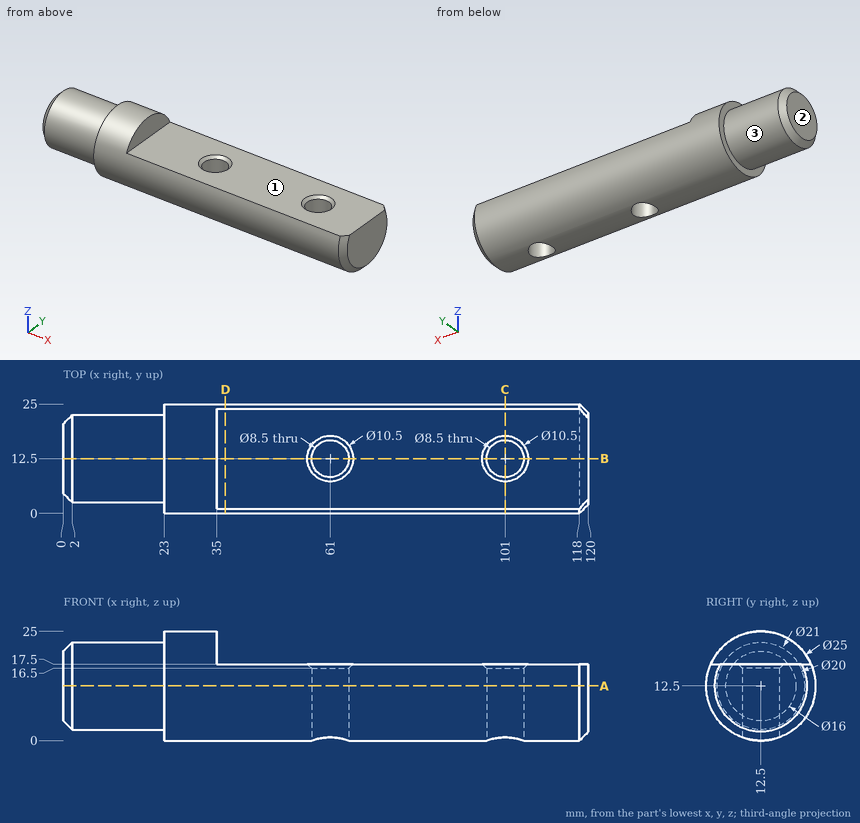
Here's the drawing with two shaded views (mm, measured from the low corner). I have some questions. A direction names the side the tool comes from. Coordinates: 2 decimals unless noted, no trailing zeros. Write each loop counter-clockwise with the first axis right and the second up, starting at its lowest first coordinate (ties: lowest second). Pieces come first, ordered by that corner, then holes. Notation, with made-up numbers: M -34,35.5 L -16,35.5 A24 cw -16,68.5 Z; hole C -15.5,-21 d11. An arc over 180 degrees is marked long. Write item = value, one per line. Start each with the question number.
Q1. If we section it at D-D, the plane x = 37: Write out the boundary of the cut face in (y, z), then the cut area to 3 significant figures.
Q2. If we section it at A-A, the plane z = 12.5: Write out the boundary of the cut face in (x, y).
Q3. If we section it at C-C, the plane x = 101: Write out the boundary of the cut face in (y, z), then the cut area to 3 significant figures.
Q4. If we section it at B-B, the plane y = 12.5: Write out the boundary of the cut face in (x, z), then the cut area to 3 significant figures.
Q5. I'm going to push flat-ended pins straight in: pin 1 (12 mm diameter, centred on x = 44, y = 11, fed in from +Z); pin 2 (8 mm diameter, centred on y = 12.5, z = 5.5, fed in from -X); pin 3 (2.5 mm diameter, centred on y = 11, z = 23, fed in from +X); pin 4 (3 mm diameter, centred on x = 102.5, y = 4.5, fed in from -Z). Where does each tip first touch, or does it pass through?
Q6. On a 3-axis mill with a long thin cutter (end or side, diameter ignored), from which of +Z, -Z, +X, -X, +Y, -Y can I reach the whole of each face in a straight line? I mean the marked faces 1, 2 and 3. Say none if no direction works.
Q7. If I drill on L1, parallel to X at y = 14.5, z = 4.5; L2, parallel to Y at x = 106, z = 12.75; L3, parallel to Y at x = 50.5, z = 5, over which ranges is the centre line in solid material (lowest first)? Write a range as [from, to].
Check sheet entries:
q1.outline = M 1.04,17.5 A12.5 ccw long 23.96,17.5 Z
q1.area = 367 mm²
q2.outline = M 0,4.5 L 2,2.5 L 23,2.5 L 23,0 L 118,0 L 120,2 L 120,23 L 118,25 L 23,25 L 23,22.5 L 2,22.5 L 0,20.5 Z; hole C 61,12.5 d8.5; hole C 101,12.5 d8.5
q3.outline = M 1.04,17.5 A12.5 ccw 8.25,0.74 L 8.25,16.5 L 7.25,17.5 Z; M 16.75,0.74 A12.5 ccw 23.96,17.5 L 17.75,17.5 L 16.75,16.5 Z
q3.area = 219 mm²
q4.outline = M 0,4.5 L 2,2.5 L 23,2.5 L 23,0 L 56.75,0 L 56.75,16.5 L 55.75,17.5 L 35,17.5 L 35,25 L 23,25 L 23,22.5 L 2,22.5 L 0,20.5 Z; M 65.25,0 L 96.75,0 L 96.75,16.5 L 95.75,17.5 L 66.25,17.5 L 65.25,16.5 Z; M 105.25,0 L 118,0 L 120,2 L 120,17.5 L 106.25,17.5 L 105.25,16.5 Z
q4.area = 1,940 mm²
q5.pin_1 = 17.5
q5.pin_2 = 0
q5.pin_3 = 35
q5.pin_4 = 1.82
q6.face_1 = +Z, +X, +Y, -Y
q6.face_2 = +Z, -Z, -X, +Y, -Y
q6.face_3 = -X
q7.L1 = [0.25, 57.25], [64.75, 97.25], [104.75, 120]
q7.L2 = [0, 25]
q7.L3 = [2.5, 22.5]
